Design review of the part shown in the three views and the two pictorial views. Dimensions are in mm from the part's minimum x, y and z. Coordinates: 2 decimals unless noted, no trailing zeros. Write each loop counter-clockwise with the first axis right and the second up, starting at its lowest first coordinate (ties: lowest second). Pieces come first, ordered by that corner, then holes. Notation, with made-up numbers: (-37, 21.5) - (-2, 21.5) arc R17 cw to (-2, 41.5) - close; hole circle Ø9 at (-33.5, 74). An arc over 180 degrees is marked (long way). Write each question's results on one line, items separated by ' | '.
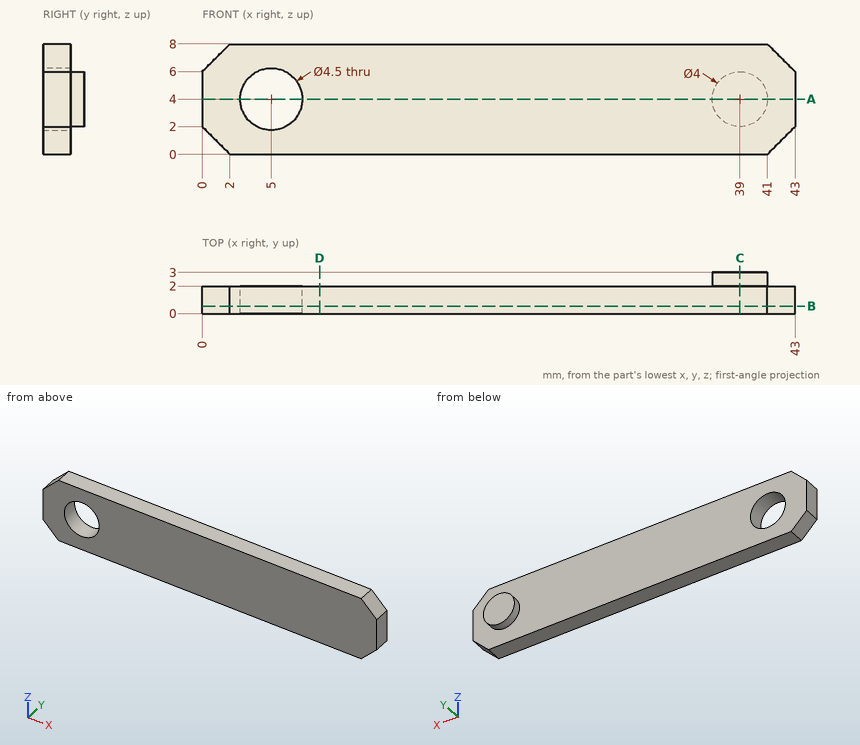
Q1. Take a section at D-D on x = 8.5. State the section outline as (y, z) points, plus the area to 3 significant figures.
Results found:
outline: (0, 0) - (2, 0) - (2, 8) - (0, 8) - close | area: 16.0 mm2
Q2. Take a section at B-B on y = 0.55. State the section outline as (x, z) points.
Results found:
outline: (0, 2) - (2, 0) - (41, 0) - (43, 2) - (43, 6) - (41, 8) - (2, 8) - (0, 6) - close; hole circle Ø4.5 at (5, 4)
Q3. For pin 1 (1.5 mm diameter, centred on x = 22.5, z = 6.5, fed in from +Y), flat-tipped, find the tip position at first contact; note if it passes through.
Results found:
pin 1: y = 2
Q4. Take a section at C-C on x = 39. State the section outline as (y, z) points.
Results found:
outline: (0, 0) - (2, 0) - (2, 2) - (3, 2) - (3, 6) - (2, 6) - (2, 8) - (0, 8) - close
Q5. Wall thickness on line 1 along X through (y, z) = (0.55, 4); line 2 along Y through (x, z) = (7.5, 7.5); line 3 along Z through (x, y) = (6, 1.3): over which ranges is each line inside the solid? List them lowest first. Write a range as from..to.
Results found:
line 1: 0..2.75, 7.25..43 | line 2: 0..2 | line 3: 0..1.98, 6.02..8
Q6. Take a section at A-A on z = 4. State the section outline as (x, y) points.
Results found:
outline: (0, 0) - (2.75, 0) - (2.75, 2) - (0, 2) - close; (7.25, 0) - (43, 0) - (43, 2) - (41, 2) - (41, 3) - (37, 3) - (37, 2) - (7.25, 2) - close
